Geometry: final body of the model. Coordinates: model frame, mm. Face numbers are marked on the shaded views. A direction names the side the tool comes from. Coordinates: 2 decimals unless noted, no trailing zeros. Write each loop counter-clockwise with the first axis right and the second up, starting at its lowest first coordinate (ties: lowest second). Pieces come first, ordered by that corner, then holes. Notation, with made-up numbers: (3, 2) -> (48, 2) arc R16 ccw to (48, 23) -> close; hole circle Ø11 at (67.5, 27.25). An arc over 180 degrees is marked (long way). Answer as a JSON object with one key per item and string values. Group by question number.
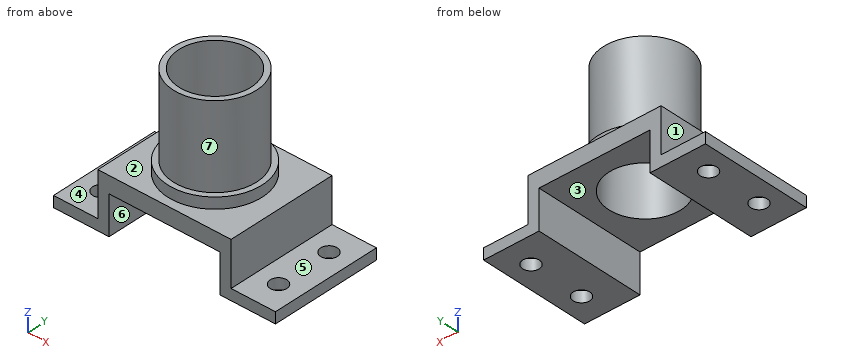
```python
from build123d import *

# Parameters (mm, degrees)
SKETCH1_R           = 7.5
SKETCH1_R_2         = 6.5
BOSS_EXTRUDE1_DEPTH = 22
BOSS_EXTRUDE2_START = 2
SKETCH2_R           = 8.5
SKETCH2_R_2         = 7.5
BOSS_EXTRUDE2_DEPTH = 2
BOSS_EXTRUDE4_START = 2
SKETCH5_R           = 7.5
SKETCH5_R_2         = 6.5
BOSS_EXTRUDE4_DEPTH = 2
BOSS_EXTRUDE5_START = 2
SKETCH6_R           = 8.5
SKETCH6_R_2         = 6.5
BOSS_EXTRUDE5_DEPTH = 2
SKETCH7_W           = 30
SKETCH7_H           = 20
BOSS_EXTRUDE6_DEPTH = 10
SKETCH8_W           = 20
SKETCH8_H           = 7
CUT_EXTRUDE1_DEPTH  = 34.301651611
SKETCH9_W           = 5
SKETCH9_H           = 20
BOSS_EXTRUDE7_DEPTH = 2
SKETCH12_R          = 6.5
CUT_EXTRUDE3_DEPTH  = 31
SKETCH13_W          = 3
SKETCH13_H          = 20
CUT_EXTRUDE4_DEPTH  = 8
SKETCH11_R          = 1.5
CUT_EXTRUDE2_DEPTH  = 34.541019662


with BuildPart() as part:
    # Sketch1 → Boss-Extrude1 (new body)
    with BuildSketch(Plane.XY):
        Circle(SKETCH1_R)
        Circle(SKETCH1_R_2, mode=Mode.SUBTRACT)
    extrude(amount=BOSS_EXTRUDE1_DEPTH)

    # Sketch2 → Boss-Extrude2 (add)
    with BuildSketch(Plane(origin=(0, 0, 7), x_dir=(-1, 0, 0), z_dir=(0, 0, -1)).offset(BOSS_EXTRUDE2_START)):
        Circle(SKETCH2_R)
        Circle(SKETCH2_R_2, mode=Mode.SUBTRACT)
    extrude(amount=-BOSS_EXTRUDE2_DEPTH)

    # Sketch5 → Boss-Extrude4 (add)
    with BuildSketch(Plane(origin=(0, 0, 0), x_dir=(-1, 0, 0), z_dir=(0, 0, -1)).offset(BOSS_EXTRUDE4_START)):
        Circle(SKETCH5_R)
        Circle(SKETCH5_R_2, mode=Mode.SUBTRACT)
    extrude(amount=-BOSS_EXTRUDE4_DEPTH)

    # Sketch6 → Boss-Extrude5 (add)
    with BuildSketch(Plane(origin=(0, 0, -2), x_dir=(-1, 0, 0), z_dir=(0, 0, -1)).offset(BOSS_EXTRUDE5_START)):
        Circle(SKETCH6_R)
        Circle(SKETCH6_R_2, mode=Mode.SUBTRACT)
    extrude(amount=-BOSS_EXTRUDE5_DEPTH)

    # Sketch7 → Boss-Extrude6 (add)
    with BuildSketch(Plane(origin=(0, 0, 5), x_dir=(-1, 0, 0), z_dir=(0, 0, -1))):
        Rectangle(SKETCH7_W, SKETCH7_H)
    extrude(amount=BOSS_EXTRUDE6_DEPTH)

    # Sketch8 → Cut-Extrude1 (cut, through all)
    with BuildSketch(Plane.XZ.offset(10)):
        with Locations((0, -1.5)):
            Rectangle(SKETCH8_W, SKETCH8_H)
    extrude(amount=-CUT_EXTRUDE1_DEPTH, mode=Mode.SUBTRACT)

    # Sketch9 → Boss-Extrude7 (add)
    with BuildSketch(Plane(origin=(0, 0, -5), x_dir=(-1, 0, 0), z_dir=(0, 0, -1))):
        with Locations((-17.5, 0)):
            Rectangle(SKETCH9_W, SKETCH9_H)
        with Locations((17.5, 0)):
            Rectangle(SKETCH9_W, SKETCH9_H)
    extrude(amount=-BOSS_EXTRUDE7_DEPTH)

    # Sketch12 → Cut-Extrude3 (cut, through all)
    with BuildSketch(Plane(origin=(0, 0, 2), x_dir=(-1, 0, 0), z_dir=(0, 0, -1))):
        Circle(SKETCH12_R)
    extrude(amount=-CUT_EXTRUDE3_DEPTH, mode=Mode.SUBTRACT)

    # Sketch13 → Cut-Extrude4 (cut)
    with BuildSketch(Plane.XY.offset(5)):
        with Locations((-13.5, 0)):
            Rectangle(SKETCH13_W, SKETCH13_H)
        with Locations((13.5, 0)):
            Rectangle(SKETCH13_W, SKETCH13_H)
    extrude(amount=-CUT_EXTRUDE4_DEPTH, mode=Mode.SUBTRACT)

    # Sketch11 → Cut-Extrude2 (cut, through all)
    with BuildSketch(Plane.XY.offset(-3)):
        with Locations((16, 5)):
            Circle(SKETCH11_R)
        with Locations((16, -5)):
            Circle(SKETCH11_R)
        with Locations(Location((-16, -5, 0), (0, 0, 180))):
            Circle(SKETCH11_R)
        with Locations(Location((-16, 5, 0), (0, 0, 180))):
            Circle(SKETCH11_R)
    extrude(amount=-CUT_EXTRUDE2_DEPTH, mode=Mode.SUBTRACT)


solid = part.part
```
Item 1: Set-up query: the marked faces 4, 5, 6 and 7. Return all of +Z, -Z, +X, -X, +Y, -Y with unobstructed straight access to the full face (end or side cutting, diameter ignored); none if empty.
Item 2: Contact query for flat-ended pins moving along their axis: pin 1 (2 mm diameter, centred on y = -1, z = 0, fed in from +X); pin 2 (6.5 mm diameter, centred on x = -14.5, y = 3, fed in from +Z); pin 3 (2.5 mm diameter, centred on x = 18, y = 1.5, fed in from +Z). Output: stop coordinate, or through.
Item 3: Section D-D on x = 0. Output: boundary loops of the cut face in (y, z), then the cut area to 3 significant figures.
Item 4: Mould query, pull axis X, two halves, no side actions, for the marked faces 1, 2 and 3. Classes: +X half, -X half, draft (parallel to the pull), parting line (faces both ways), or undercut.
Item 5: Section C-C on z = 0.5. Output: boundary loops of the cut face in (x, y).
Item 6: Ray query, L1, parallel to Y at x = 16, z = -4.2; L2, parallel to X at y = 0, z = 8. Return the intervals inside material, ascending. Write a range as [from, to].
Item 7: Section B-B on y = 0. Output: boundary loops of the cut face in (x, z), then the cut area to 3 significant figures.
Item 8: Section A-A on x = 16. Output: boundary loops of the cut face in (y, z), then the cut area to 3 significant figures.
Answer sheet:
{
 "1": {"face 4": "+Z, -X, +Y, -Y", "face 5": "+Z, +X, +Y, -Y", "face 6": "-Z, +Y, -Y", "face 7": "+Z"},
 "2": {"pin 1": "stops at x = 12", "pin 2": "stops at z = 5", "pin 3": "stops at z = -3"},
 "3": {"outline": "(-10, 2) -> (-6.5, 2) -> (-6.5, 22) -> (-7.5, 22) -> (-7.5, 7) -> (-8.5, 7) -> (-8.5, 5) -> (-10, 5) -> close; (6.5, 2) -> (10, 2) -> (10, 5) -> (8.5, 5) -> (8.5, 7) -> (7.5, 7) -> (7.5, 22) -> (6.5, 22) -> close", "area": "59.0 mm^2"},
 "4": {"face 1": "-X half", "face 2": "draft", "face 3": "undercut"},
 "5": {"outline": "(-12, -10) -> (-10, -10) -> (-10, 10) -> (-12, 10) -> close; (10, -10) -> (12, -10) -> (12, 10) -> (10, 10) -> close"},
 "6": {"L1": "y = [-10, -6.5], [-3.5, 3.5], [6.5, 10]", "L2": "x = [-7.5, -6.5], [6.5, 7.5]"},
 "7": {"outline": "(-20, -5) -> (-10, -5) -> (-10, 2) -> (-6.5, 2) -> (-6.5, 22) -> (-7.5, 22) -> (-7.5, 7) -> (-8.5, 7) -> (-8.5, 5) -> (-12, 5) -> (-12, -3) -> (-20, -3) -> close; (6.5, 2) -> (10, 2) -> (10, -5) -> (20, -5) -> (20, -3) -> (12, -3) -> (12, 5) -> (8.5, 5) -> (8.5, 7) -> (7.5, 7) -> (7.5, 22) -> (6.5, 22) -> close", "area": "131 mm^2"},
 "8": {"outline": "(-10, -5) -> (-6.5, -5) -> (-6.5, -3) -> (-10, -3) -> close; (-3.5, -5) -> (3.5, -5) -> (3.5, -3) -> (-3.5, -3) -> close; (6.5, -5) -> (10, -5) -> (10, -3) -> (6.5, -3) -> close", "area": "28.0 mm^2"}
}
